```python
from build123d import *

# Parameters (mm, degrees)
BORE_13_DEPTH                     = 73.608539443
BORE_13_DEPTH_BACK                = 73.608539443
BORE_13_SKETCH_R                  = 8
RECESS_START                      = 10
RECESS_15_SKETCH_R                = 7.5
RECESS_15X10_DEPTH                = 63.608539443
COUNTERBORE_START                 = 12
COUNTERBORE_18_SKETCH_R           = 9
COUNTERBORE_18X12_DEPTH           = 61.608539443
HANDLE_SHANK_BORE_10_2_DEPTH      = 73.608539443
HANDLE_SHANK_BORE_10_2_DEPTH_BACK = 73.608539443
SKETCH6_R                         = 5.1


with BuildPart() as part:
    # Handle Profile Sketch → Handle Body Revolve (revolve)
    with BuildSketch(Plane.XY):
        with BuildLine():
            Line((-31.583592135, 12), (-10.988504472, 10.210424549))
            ThreePointArc((-10.988504472, 10.210424549), (1.298506798, 14.943690311), (12.58494961, 8.162048965))
            Line((12.58494961, 8.162048965), (43.220781011, 5.5))
            ThreePointArc((43.220781011, 5.5), (57.816926795, 12.691135624), (68, 0))
            Line((68, 0), (-63, 0))
            ThreePointArc((-63, 0), (-51.422797616, 16.815102461), (-31.583592135, 12))
        make_face()
    revolve(axis=Axis((-65.491317505, 0, 0), (1, 0, 0)))

    # Bore Ø13 Sketch → Bore Ø13 (cut, two sides: drawn at the far end of the back side and taken through both)
    with BuildSketch(Plane(origin=(0, 0, 0), x_dir=(1, 0, 0), z_dir=(0, 1, 0)).offset(-BORE_13_DEPTH_BACK)):
        with Locations(Location((0, 0, 0), (0, 0, 270))):
            Circle(BORE_13_SKETCH_R)
    extrude(amount=BORE_13_DEPTH + BORE_13_DEPTH_BACK, mode=Mode.SUBTRACT)

    # Recess Ø15 Sketch → Recess Ø15x10 (cut, through all)
    with BuildSketch(Plane(origin=(0, 0, 0), x_dir=(1, 0, 0), z_dir=(0, 1, 0)).offset(RECESS_START)):
        with Locations(Location((55, 0, 0), (0, 0, 90))):
            Circle(RECESS_15_SKETCH_R)
    extrude(amount=RECESS_15X10_DEPTH, mode=Mode.SUBTRACT)

    # Counterbore Ø18 Sketch → Counterbore Ø18x12 (cut, through all)
    with BuildSketch(Plane(origin=(0, 0, 0), x_dir=(1, 0, 0), z_dir=(0, 1, 0)).offset(COUNTERBORE_START)):
        Circle(COUNTERBORE_18_SKETCH_R)
    counterbore_18x12 = extrude(amount=COUNTERBORE_18X12_DEPTH, mode=Mode.SUBTRACT)

    # Counterbore Mirror: Counterbore Ø18x12 across plane
    add(counterbore_18x12.mirror(Plane.ZX), mode=Mode.SUBTRACT)

    # Sketch6 → Handle Shank Bore Ø10.2 (cut, two sides: drawn at the far end of the back side and taken through both)
    with BuildSketch(Plane(origin=(0, 0, 0), x_dir=(1, 0, 0), z_dir=(0, 1, 0)).offset(-HANDLE_SHANK_BORE_10_2_DEPTH_BACK)):
        with Locations(Location((55, 0, 0), (0, 0, 270))):
            Circle(SKETCH6_R)
    extrude(amount=HANDLE_SHANK_BORE_10_2_DEPTH + HANDLE_SHANK_BORE_10_2_DEPTH_BACK, mode=Mode.SUBTRACT)


solid = part.part
```
CAD build for the part. Positions are in the model's coordinates, mm. A direction names the side the tool comes from. Round coordinates to 2 decimals unless told otherwise and drop trailing zeros. Write each loop counter-clockwise with the first axis right and the second up, starting at its lowest first coordinate (ties: lowest second). Pieces come first, ordered by that corner, then holes.
Item 1: Drill centre lines: L1, parallel to X at y = -0.5, z = 0; L2, parallel to Z at x = 55, y = 0.5; L3, parallel to X at y = 3.5, z = 0. Where is each one in solid material? Low to high.
Filled in:
L1: x = -62.99 to -8, 8 to 49.9, 60.1 to 67.99
L2: z = -12.99 to -5.1, 5.1 to 12.99
L3: x = -62.66 to -8, 8 to 49.9, 60.1 to 67.52
Item 2: Band-saw the part on B-B on x = 0. Write the cut outline in (y, z), then the cut area to 3 significant figures.
Filled in:
outline: (-12, -9) arc R15 ccw to (12, -9) - (12, -8) - (-12, -8) - close; (-12, 8) - (12, 8) - (12, 9) arc R15 ccw to (-12, 9) - close
area: 249 mm2
Item 3: Band-saw the part on C-C on z = 0. Write the cut outline in (x, y), then the cut area to 3 significant figures.
Filled in:
outline: (-31.58, -12) - (-10.99, -10.21) arc R15 ccw to (-9, -12) - (-8, -12) - (-8, 12) - (-9, 12) arc R15 ccw to (-10.99, 10.21) - (-31.58, 12) arc R18 ccw (long way) to start; (8, -12) - (9, -12) arc R15 ccw to (12.58, -8.16) - (43.22, -5.5) arc R13 ccw to (49.9, -11.96) - (49.9, 10) - (47.5, 10) - (47.5, 10.62) arc R13 ccw to (43.22, 5.5) - (12.58, 8.16) arc R15 ccw to (9, 12) - (8, 12) - close; (60.1, -11.96) arc R13 ccw to (62.5, 10.62) - (62.5, 10) - (60.1, 10) - close
area: 2,240 mm2
Item 4: Tool access for faces 1 (the cylindrical face through (60, -1, -1)), 2 (the conical face through (-21.14, -2.4, -10.83)), 3 (the flat face through (57, 10, -5)): list every direction of +Z, -Z, +X, -X, +Y, -Y with a clear straight run to the whole face (end or side of a thin tool).
Filled in:
face 1: +Y, -Y
face 2: none
face 3: +Y
Item 5: Band-saw the part on A-A on x = 55. Write the cut outline in (y, z).
Filled in:
outline: (-11.96, -5.1) arc R13 ccw to (10.62, -7.5) - (10, -7.5) - (10, -5.1) - close; (-11.96, 5.1) - (10, 5.1) - (10, 7.5) - (10.62, 7.5) arc R13 ccw to start
Item 6: Drop flat-ended pins along their axis: pin 1 Ø16.5 at (x, z) = (53.5, -3) entering from +Y; pin 2 Ø8 at (x, y) = (-37.5, -12.5) entering from +Z; pin 3 Ø1.5 at (x, y) = (-40.5, 3.5) entering from +Z. Give the stop position or say it passes through.
Filled in:
pin 1: stops at y = 10.62
pin 2: stops at z = 14.56
pin 3: stops at z = 17.31
Item 7: Band-saw the part on D-D on y = 7. Give the number of separate pieces and of enclosed holes in the cut face, then the cut area to 3 significant figures.
Filled in:
separate pieces: 2
enclosed holes: 2
area: 1,870 mm2
